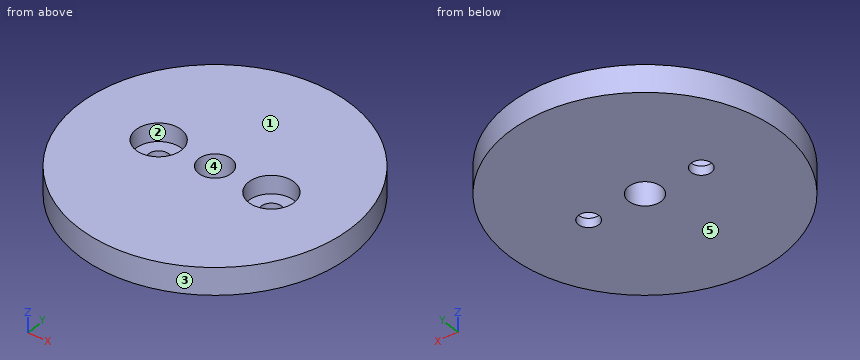
```python
from build123d import *

# Parameters (mm, degrees)
SKETCH1_R                               = 30
BOSS_EXTRUDE1_DEPTH                     = 6
CBORE_FOR_M4_HEX_HEAD_BOLT1_D           = 4.5
CBORE_FOR_M4_HEX_HEAD_BOLT1_CBORE_D     = 10
CBORE_FOR_M4_HEX_HEAD_BOLT1_CBORE_DEPTH = 4
SKETCH4_R                               = 3.6
CUT_EXTRUDE1_DEPTH                      = 10


with BuildPart() as part:
    # Sketch1 → Boss-Extrude1 (new body)
    with BuildSketch(Plane.XY):
        Circle(SKETCH1_R)
    extrude(amount=BOSS_EXTRUDE1_DEPTH)

    # CBORE for M4 Hex Head Bolt1 (through all)
    with Locations(Plane.XY.offset(6)):
        with Locations((-12.5, 0), (12.5, 0)):
            CounterBoreHole(CBORE_FOR_M4_HEX_HEAD_BOLT1_D / 2, CBORE_FOR_M4_HEX_HEAD_BOLT1_CBORE_D / 2, CBORE_FOR_M4_HEX_HEAD_BOLT1_CBORE_DEPTH)

    # Sketch4 → Cut-Extrude1 (cut)
    with BuildSketch(Plane.XY.offset(6)):
        Circle(SKETCH4_R)
    extrude(amount=-CUT_EXTRUDE1_DEPTH, mode=Mode.SUBTRACT)


solid = part.part
```
Here's how the part is built. I have some questions about the finished solid (model axes, mm). Face numbers are marked on the shaded views. A direction names the side the tool comes from. Give positions to 0.01 mm unless a question says otherwise; leave off trailing zeros. Loops run counter-clockwise (first coordinate to the right, second up) from the corner with the lowest first, then second, coordinate; pieces in that order, holes last. Notation, with made-up numbers: M 24.5,57.25 L 55.5,57.25 A32 ccw 55.5,93.25 Z; hole C -5.75,13 d7. An arc over 180 degrees is marked long. Put each result on its own line as item: value. Start each with the question number.
(1) Will these pins go through, and if not, where does the flat tip stop? pin 1 Ø3.5 at (x, y) = (-12.5, 0) entering from -Z; pin 2 Ø3 at (y, z) = (16, 4.5) entering from -X; pin 3 Ø1.5 at (x, z) = (-16, 3) entering from +Y; pin 4 Ø3 at (x, y) = (-12, -1.5) entering from +Z.
(2) For the marked faces 1 and 2, which set-ups out of +Z, -Z, +X, -X, +Y, -Y let a thin tool reach every point of the face, with its end or its side?
(3) I want a section at B-B on y = 0. Please give me the cut outline in (x, z).
(4) If we mould it in two halves opening along X, with no side actions, what happens to the marked faces 3, 4 and 5? For each: +X half, -X half, draft (parallel to the pull), parting line (faces both ways), or undercut.
(5) I want a section at C-C on z = 1.2. Please give me the cut outline in (x, y), then the cut area to 3 significant figures.
(6) I want a section at A-A on x = 0. Please give me the cut outline in (y, z), then the cut area to 3 significant figures.
(7) I need wall thicknesses on line 1 along Y through (x, z) = (0, 4.2); line 2 along X through (y, z) = (-0.5, 1.65); line 3 along Y through (x, z) = (-12.5, 0.6). Which ranges of each line are inside material? Lowest first, please. Write a range as [from, to].
(8) I want a section at D-D on x = -12.5. Please give me the cut outline in (y, z), then the cut area to 3 significant figures.
Answer block:
1. pin 1: through
1. pin 2: x = -26.26
1. pin 3: y = 25.83
1. pin 4: z = 2
2. face 1: +Z, +X, -X, +Y, -Y
2. face 2: +Z
3. outline: M -30,0 L -14.75,0 L -14.75,2 L -17.5,2 L -17.5,6 L -30,6 Z; M -10.25,0 L -3.6,0 L -3.6,6 L -7.5,6 L -7.5,2 L -10.25,2 Z; M 3.6,0 L 10.25,0 L 10.25,2 L 7.5,2 L 7.5,6 L 3.6,6 Z; M 14.75,0 L 30,0 L 30,6 L 17.5,6 L 17.5,2 L 14.75,2 Z
4. face 3: parting line
4. face 4: undercut
4. face 5: draft
5. outline: C 0,0 d60; hole C -12.5,0 d4.5; hole C 0,0 d7.2; hole C 12.5,0 d4.5
5. area: 2,750 mm^2
6. outline: M -30,0 L -3.6,0 L -3.6,6 L -30,6 Z; M 3.6,0 L 30,0 L 30,6 L 3.6,6 Z
6. area: 317 mm^2
7. line 1: [-30, -3.6], [3.6, 30]
7. line 2: [-30, -14.69], [-10.31, -3.57], [3.57, 10.31], [14.69, 30]
7. line 3: [-27.27, -2.25], [2.25, 27.27]
8. outline: M -27.27,0 L -2.25,0 L -2.25,2 L -5,2 L -5,6 L -27.27,6 Z; M 2.25,0 L 27.27,0 L 27.27,6 L 5,6 L 5,2 L 2.25,2 Z
8. area: 278 mm^2
